```python
from build123d import *

# Parameters (mm, degrees)
SKETCH1_R               = 100
SKETCH1_R_2             = 50
BOSS_EXTRUDE1_DEPTH     = 1000
BOSS_EXTRUDE2_DEPTH     = 400
CUT_EXTRUDE2_DEPTH      = 1419.846362366
CUT_EXTRUDE2_DEPTH_BACK = 1419.846362366
CUT_EXTRUDE3_DEPTH      = 1419.846362366
CUT_EXTRUDE3_DEPTH_BACK = 1419.846362366
SKETCH_4_5_2_R          = 50


with BuildPart() as part:
    # Sketch1 → Boss-Extrude1 (new body)
    with BuildSketch(Plane(origin=(0, 0, 0), x_dir=(0, 0, -1), z_dir=(1, 0, 0))):
        Circle(SKETCH1_R)
        Circle(SKETCH1_R_2, mode=Mode.SUBTRACT)
    extrude(amount=BOSS_EXTRUDE1_DEPTH)

    # Sketch3 → Boss-Extrude2 (add)
    with BuildSketch(Plane(origin=(1000, 0, 0), x_dir=(0, 0, -1), z_dir=(1, 0, 0))):
        with BuildLine():
            Line((-75, 129.903810568), (-75, -129.903810568))
            ThreePointArc((-75, -129.903810568), (0, -150), (75, -129.903810568))
            Line((75, -129.903810568), (75, 129.903810568))
            ThreePointArc((75, 129.903810568), (0, 150), (-75, 129.903810568))
        make_face()
    extrude(amount=BOSS_EXTRUDE2_DEPTH)

    # Sketch 4_5 → Cut-Extrude2 (cut, two sides: drawn at the far end of the back side and taken through both)
    with BuildSketch(Plane.XY.offset(75).offset(-CUT_EXTRUDE2_DEPTH_BACK)):
        with BuildLine():
            Line((1250, 150), (1455.357524725, 150))
            Line((1455.357524725, 150), (1455.357524725, -150))
            Line((1455.357524725, -150), (1250, -150))
            ThreePointArc((1250, -150), (1400, 0), (1250, 150))
        make_face()
    extrude(amount=CUT_EXTRUDE2_DEPTH + CUT_EXTRUDE2_DEPTH_BACK, mode=Mode.SUBTRACT)

    # Sketch 4_5 2 → Cut-Extrude3 (cut, two sides: drawn at the far end of the back side and taken through both)
    with BuildSketch(Plane.XY.offset(75).offset(-CUT_EXTRUDE3_DEPTH_BACK)):
        with Locations((1250, 0)):
            Circle(SKETCH_4_5_2_R)
    extrude(amount=CUT_EXTRUDE3_DEPTH + CUT_EXTRUDE3_DEPTH_BACK, mode=Mode.SUBTRACT)


solid = part.part
```
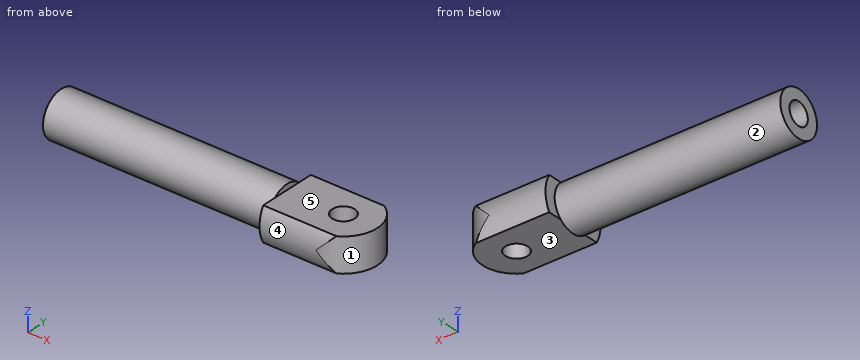
Build history of the part. All positions in model axes, mm. Face numbers are marked on the shaded views. A direction names the side the tool comes from. Round coordinates to 2 decimals unless told otherwise and drop trailing zeros. Write each loop counter-clockwise with the first axis right and the second up, starting at its lowest first coordinate (ties: lowest second). Pieces come first, ordered by that corner, then holes.
1) Band-saw the part on A-A, the plane y = 0. List the corners of the cut face in (x, z).
2) Band-saw the part on C-C, the plane x = 343. List the corners of the cut face in (y, z).
3) Pin check, flat tips, straight feed: pin 1 (5 mm diameter, centred on x = 252.5, y = 70.5, fed in from -Z); pin 2 (6 mm diameter, centred on x = 588, z = -12.5, fed in from +Y); pin 3 (12.5 mm diameter, centred on y = -1, z = 90, fed in from +X); pin 4 (8 mm diameter, centred on y = -64, z = 48, fed in from -X). Stop position of each tip, or through.
4) Band-saw the part on B-B, the plane z = 0. List the corners of the cut face in (x, y).
5) Band-saw the part on D-D, the plane y = 86. List the corners of the cut face in (x, z).
6) Drill centre lines: probe 1 along Y at (x, z) = (290, 0); probe 2 along Y at (x, z) = (1250, 43); probe 3 along Z at (x, y) = (739.5, 40). Where is each one in solid material? Low to high.
7) 3-axis set-ups, long thin cutter, end or side, ignore diameter. For the marked faces 1, 2, 3, 4 and 5: which of +Z, -Z, +X, -X, +Y, -Y reach the whole face in a straight line?
Ans:
1. outline: (0, -100) - (1000, -100) - (1000, -75) - (1200, -75) - (1200, 75) - (1000, 75) - (1000, 100) - (0, 100) - (0, 50) - (1000, 50) - (1000, -50) - (0, -50) - close; (1300, -75) - (1400, -75) - (1400, 75) - (1300, 75) - close
2. outline: circle Ø200 at (0, 0); hole circle Ø100 at (0, 0)
3. pin 1: stops at z = -73.32
3. pin 2: stops at y = 99.55
3. pin 3: stops at x = 1000
3. pin 4: stops at x = 0
4. outline: (0, -100) - (1000, -100) - (1000, -150) - (1250, -150) arc R150 ccw to (1250, 150) - (1000, 150) - (1000, 100) - (0, 100) - (0, 50) - (1000, 50) - (1000, -50) - (0, -50) - close; hole circle Ø100 at (1250, 0)
5. outline: (0, -51.03) - (1000, -51.03) - (1000, -75) - (1372.9, -75) - (1372.9, 75) - (1000, 75) - (1000, 51.03) - (0, 51.03) - close
6. probe 1: y = -100 to -50, 50 to 100
6. probe 2: y = -143.7 to -50, 50 to 143.7
6. probe 3: z = -91.65 to -30, 30 to 91.65
7. face 1: +Z, -Z, +X
7. face 2: -X
7. face 3: -Z, +X, +Y, -Y
7. face 4: +X, -X, -Y
7. face 5: +Z, +X, +Y, -Y
